Verification items for the finished model (mm, model axes). Face numbers are marked on the shaded views. A direction names the side the tool comes from. Give positions to 0.01 mm unless a question says otherwise; leave off trailing zeros. Order: outer loops, then holes, each group sorted by start corner. A loop starts at its lowest first (then second) coordinate and runs counter-clockwise, first axis right, second up. Notation, with made-up numbers: M 67.25,-32.75 L 80.25,-32.75 A5 cw 80.25,-26.75 Z; hole C 38.25,41 d5. An arc over 180 degrees is marked long. Answer as a JSON object with one key per item and string values.
```python
from build123d import *

# Parameters (mm, degrees)
ROD_PROFILE_SKETCH_R   = 8
ROD_PROFILE_SKETCH_R_2 = 13
ROD_BODY_10MM_DEPTH    = 5
WEB_RECESS_1_5MM_DEPTH = 0.75


with BuildPart() as part:
    # Rod Profile Sketch → Rod Body 10mm (new, symmetric)
    with BuildSketch(Plane.XY):
        with BuildLine():
            Line((-12.462962882, 65.961538462), (-22.433333187, -63.269230769))
            ThreePointArc((-22.433333187, -63.269230769), (0, -87.5), (22.433333187, -63.269230769))
            Line((22.433333187, -63.269230769), (12.462962882, 65.961538462))
            ThreePointArc((12.462962882, 65.961538462), (0, 77.5), (-12.462962882, 65.961538462))
        make_face()
        with Locations((0, 65)):
            Circle(ROD_PROFILE_SKETCH_R, mode=Mode.SUBTRACT)
        with Locations((0, -65)):
            Circle(ROD_PROFILE_SKETCH_R_2, mode=Mode.SUBTRACT)
        with BuildLine():
            Line((-8.247008498, 55.606552772), (-16.360291448, -49.553613246))
            ThreePointArc((-16.360291448, -49.553613246), (0, -42.5), (16.360291448, -49.553613246))
            Line((16.360291448, -49.553613246), (8.247008498, 55.606552772))
            ThreePointArc((8.247008498, 55.606552772), (0, 52.5), (-8.247008498, 55.606552772))
        make_face(mode=Mode.SUBTRACT)
    extrude(amount=ROD_BODY_10MM_DEPTH, both=True)

    # Sketch1_3 → Web Recess 1.5mm (add, symmetric)
    with BuildSketch(Plane.XY):
        with BuildLine():
            ThreePointArc((16.360291448, -49.553613246), (0, -42.5), (-16.360291448, -49.553613246))
            Line((-16.360291448, -49.553613246), (-8.247008498, 55.606552772))
            ThreePointArc((-8.247008498, 55.606552772), (0, 52.5), (8.247008498, 55.606552772))
            Line((8.247008498, 55.606552772), (16.360291448, -49.553613246))
        make_face()
    extrude(amount=WEB_RECESS_1_5MM_DEPTH, both=True)


solid = part.part
```
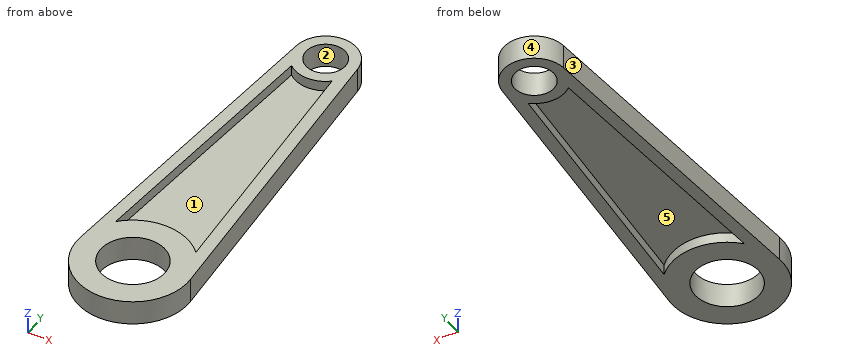
Q1. Material ranges on L1, parallel to Y at x = -4.5, z = -2; L2, parallel to X at y = 54.5, z = -4.5; L3, parallel to X at y = -6, z = 4.5, recorded low to high.
Resolved:
{"L1": "y = -87.05 to -77.2, -52.8 to -42.95, 53.34 to 58.39, 71.61 to 76.66", "L2": "x = -13.35 to -8.33, -6.78 to 6.78, 8.33 to 13.35", "L3": "x = -18.01 to -13, 13 to 18.01"}
Q2. Gauge pin test, flat ends, axial feed: pin 1 Ø1.5 at (x, z) = (5.5, 0.5) entering from +Y; pin 2 Ø16.5 at (x, y) = (2, 21.5) entering from +Z; pin 3 Ø3 at (y, z) = (-43, 0) entering from -X; pin 4 Ø9.5 at (x, y) = (0, 65) entering from -Z. Record the tip position at first contact, or that the pin passes through.
Resolved:
{"pin 1": "stops at y = 76.56", "pin 2": "stops at z = 0.75", "pin 3": "stops at x = -20.99", "pin 4": "passes through"}
Q3. Tool access check on the marked faces 1 and 2. Record the directions out of +Z, -Z, +X, -X, +Y, -Y that give a thin tool (end or side, any length) a straight path to the whole face; none if there is none.
Resolved:
{"face 1": "+Z", "face 2": "+Z, -Z"}
Q4. Section check D-D on y = 15.5. Record the cut outline in (x, z), then the cut area to 3 significant figures.
Resolved:
{"outline": "M -16.36,-5 L -11.34,-5 L -11.34,-0.75 L 11.34,-0.75 L 11.34,-5 L 16.36,-5 L 16.36,5 L 11.34,5 L 11.34,0.75 L -11.34,0.75 L -11.34,5 L -16.36,5 Z", "area": "134 mm²"}
Q5. Section check B-B on x = 0. Record the cut outline in (y, z), then the cut area to 4 significant figures.
Resolved:
{"outline": "M -87.5,-5 L -78,-5 L -78,5 L -87.5,5 Z; M -52,-5 L -42.5,-5 L -42.5,-0.75 L 52.5,-0.75 L 52.5,-5 L 57,-5 L 57,5 L 52.5,5 L 52.5,0.75 L -42.5,0.75 L -42.5,5 L -52,5 Z; M 73,-5 L 77.5,-5 L 77.5,5 L 73,5 Z", "area": "422.5 mm²"}
Q6. Section check C-C on x = 10. Record the cut outline in (y, z), then the cut area to 3 significant figures.
Resolved:
{"outline": "M -85.16,-5 L -73.31,-5 L -73.31,5 L -85.16,5 Z; M -56.69,-5 L -44.84,-5 L -44.84,-0.75 L 32.89,-0.75 L 32.89,-5 L 72.5,-5 L 72.5,5 L 32.89,5 L 32.89,0.75 L -44.84,0.75 L -44.84,5 L -56.69,5 Z", "area": "750 mm²"}
Q7. Release check for a two-part mould opening along X. For the marked faces 3, 4 and 5 record: +X half, -X half, draft (parallel to the pull), parting line (faces both ways), or undercut.
Resolved:
{"face 3": "-X half", "face 4": "parting line", "face 5": "undercut"}
Q8. Section check A-A on y = -65. Record the cut outline in (x, z).
Resolved:
{"outline": "M -22.5,-5 L -13,-5 L -13,5 L -22.5,5 Z; M 13,-5 L 22.5,-5 L 22.5,5 L 13,5 Z"}
